```python
from build123d import *

# Parameters (mm, degrees)
BOSS_EXTRUDE2_DEPTH = 200
CUT_EXTRUDE1_DEPTH  = 200
SKETCH3_R           = 3.5
CUT_EXTRUDE2_DEPTH  = 200
CUT_EXTRUDE3_DEPTH  = 10


with BuildPart() as part:
    # Sketch1 → Boss-Extrude2 (new body)
    with BuildSketch(Plane.XY):
        with BuildLine():
            Line((0, 0), (0, 160))
            ThreePointArc((0, 160), (2.928932188, 167.071067812), (10, 170))
            Line((10, 170), (190, 170))
            ThreePointArc((190, 170), (197.071067812, 167.071067812), (200, 160))
            Line((200, 160), (200, 0))
            Line((200, 0), (194, 0))
            Line((194, 0), (194, 160))
            ThreePointArc((194, 160), (192.828427125, 162.828427125), (190, 164))
            Line((190, 164), (10, 164))
            ThreePointArc((10, 164), (7.171572875, 162.828427125), (6, 160))
            Line((6, 160), (6, 0))
            Line((6, 0), (0, 0))
        make_face()
    extrude(amount=BOSS_EXTRUDE2_DEPTH)

    # Sketch2 → Cut-Extrude1 (cut)
    with BuildSketch(Plane(origin=(200, 0, 0), x_dir=(0, 0, -1), z_dir=(1, 0, 0))):
        Polygon((-200, 120), (-65, 0), (-50, 0), (-50, 100), (0, 100), (0, -9.162692683), (-225.149686355, -7.960981017), (-227.038090402, 77.768418596), align=None)
    extrude(amount=-CUT_EXTRUDE1_DEPTH, mode=Mode.SUBTRACT)

    # Sketch3 → Cut-Extrude2 (cut)
    with BuildSketch(Plane(origin=(200, 0, 0), x_dir=(0, 0, -1), z_dir=(1, 0, 0))):
        with Locations(Location((-170, 135, 0), (0, 0, 90))):
            Circle(SKETCH3_R)
        with Locations(Location((-110, 135, 0), (0, 0, 90))):
            Circle(SKETCH3_R)
    extrude(amount=-CUT_EXTRUDE2_DEPTH, mode=Mode.SUBTRACT)

    # Sketch4 → Cut-Extrude3 (cut)
    with BuildSketch(Plane(origin=(0, 170, 0), x_dir=(1, 0, 0), z_dir=(0, 1, 0))):
        with BuildLine():
            Line((165, -25), (145, -25))
            ThreePointArc((145, -25), (140, -20), (145, -15))
            Line((145, -15), (165, -15))
            ThreePointArc((165, -15), (170, -20), (165, -25))
        make_face()
        with BuildLine():
            Line((165, -155), (145, -155))
            ThreePointArc((145, -155), (140, -150), (145, -145))
            Line((145, -145), (165, -145))
            ThreePointArc((165, -145), (170, -150), (165, -155))
        make_face()
        with BuildLine():
            Line((55, -25), (35, -25))
            ThreePointArc((35, -25), (30, -20), (35, -15))
            Line((35, -15), (55, -15))
            ThreePointArc((55, -15), (60, -20), (55, -25))
        make_face()
        with BuildLine():
            Line((55, -155), (35, -155))
            ThreePointArc((35, -155), (30, -150), (35, -145))
            Line((35, -145), (55, -145))
            ThreePointArc((55, -145), (60, -150), (55, -155))
        make_face()
    extrude(amount=-CUT_EXTRUDE3_DEPTH, mode=Mode.SUBTRACT)


solid = part.part
```
Part model, mm, in its own coordinate system. A direction names the side the tool comes from. Give positions to 0.01 mm unless a question says otherwise; leave off trailing zeros. Write each loop counter-clockwise with the first axis right and the second up, starting at its lowest first coordinate (ties: lowest second). Pieces come first, ordered by that corner, then holes. Notation, with made-up numbers: M 26,88 L 80,88 A14 cw 80,92 Z; hole C 63.5,22 d3. An arc over 180 degrees is marked long. Use CSV: the item, a comma, the result in double quotes.
Item 1: Slice it at A-A on y = 155. Write the cut outline in (x, z), plus the area to 3 significant figures.
Taken from the geometry:
outline,"M 0,0 L 6,0 L 6,200 L 0,200 Z; M 194,0 L 200,0 L 200,200 L 194,200 Z"
area,"2,400 mm²"
Item 2: Slice it at C-C on z = 62. Write the cut outline in (x, y), plus the area to 3 significant figures.
Taken from the geometry:
outline,"M 0,0 L 6,0 L 6,160 A4 cw 10,164 L 190,164 A4 cw 194,160 L 194,0 L 200,0 L 200,160 A10 ccw 190,170 L 10,170 A10 ccw 0,160 Z"
area,"3,130 mm²"
Item 3: Drill centre lines: probe 1 along Z at (x, y) = (198, 135); probe 2 along X at (y, z) = (98.5, 160); probe 3 along Y at (x, z) = (186, 161.5). Where is each one in solid material? Low to high.
Taken from the geometry:
probe 1,"z = 0 to 106.5, 113.5 to 166.5, 173.5 to 200"
probe 2,"x = 0 to 6, 194 to 200"
probe 3,"y = 164 to 170"
Item 4: Pin check, flat tips, straight feed: P1, Ø6.5, axis at x = 4, z = 32.5, coming from the -Y side; P2, Ø5, axis at x = 197, y = 38, coming from the -Z side. Stop position of each tip, or through.
Taken from the geometry:
P1,"stops at y = 100"
P2,"stops at z = 50"
Item 5: Pull direction X, two halves, no side cores. Call faces 3 (the face through (196.99, 167.15, 98.6)), 4 (the face through (45, 167, 25)), 5 (the face through (3.042, 138.233, 108.659)), 6 (the face through (45, 167, 155)): +X half, -X half, draft (parallel to the pull), parting line (faces both ways), or undercut.
Taken from the geometry:
face 3,"+X half"
face 4,"undercut"
face 5,"draft"
face 6,"undercut"
Item 6: Slice it at B-B on x = 151.5. Write the cut outline in (y, z).
Taken from the geometry:
outline,"M 164,0 L 170,0 L 170,15 L 164,15 Z; M 164,25 L 170,25 L 170,145 L 164,145 Z; M 164,155 L 170,155 L 170,200 L 164,200 Z"
Item 7: Slice it at D-D on z = 110. Write the cut outline in (x, y).
Taken from the geometry:
outline,"M 0,40 L 6,40 L 6,131.5 L 0,131.5 Z; M 0,138.5 L 6,138.5 L 6,160 A4 cw 10,164 L 190,164 A4 cw 194,160 L 194,138.5 L 200,138.5 L 200,160 A10 ccw 190,170 L 10,170 A10 ccw 0,160 Z; M 194,40 L 200,40 L 200,131.5 L 194,131.5 Z"
Item 8: Which spindle directions (+Z, -Z, +X, -X, +Y, -Y) get a long thin tool onto all of the face, cutting with end or side? Do faces 1 (the face through (155, 167, 155)), 2 (the face through (3.042, 138.233, 168.659)). Say none if no direction does.
Taken from the geometry:
face 1,"+Y, -Y"
face 2,"+X, -X"
